from build123d import *

# Parameters (mm, degrees)
SKETCH_2_R          = 8.5
SKETCH_2_R_2        = 8
CUT_EXTRUDE_1_DEPTH = 28
CUT_EXTRUDE_START   = 2
SKETCH_3_R          = 8
SKETCH_3_R_2        = 7
CUT_EXTRUDE_2_DEPTH = 2


with BuildPart() as part:
    # 草图1 → 旋转1 (revolve)
    with BuildSketch(Plane.XY, mode=Mode.PRIVATE) as revolve_1_sk:
        Polygon((0, 0), (0, 13), (3, 13), (3, 8.5), (70, 8.5), (70, 0), align=None)
    revolve(revolve_1_sk.sketch.rotate(Axis((0, 0, 0), (1, 0, 0)), 90), axis=Axis((0, 0, 0), (1, 0, 0)))

    # 草图2 → 切除-拉伸1 (cut)
    with BuildSketch(Plane(origin=(70, 0, 0), x_dir=(0, 0, -1), z_dir=(1, 0, 0))):
        with Locations(Location((0, 0, 0), (0, 0, 180))):
            Circle(SKETCH_2_R)
        Circle(SKETCH_2_R_2, mode=Mode.SUBTRACT)
    extrude(amount=-CUT_EXTRUDE_1_DEPTH, mode=Mode.SUBTRACT)

    # 草图3 → 切除-拉伸2 (cut)
    with BuildSketch(Plane(origin=(42, 0, 0), x_dir=(0, 0, -1), z_dir=(1, 0, 0)).offset(CUT_EXTRUDE_START)):
        Circle(SKETCH_3_R)
        Circle(SKETCH_3_R_2, mode=Mode.SUBTRACT)
    extrude(amount=-CUT_EXTRUDE_2_DEPTH, mode=Mode.SUBTRACT)


solid = part.part
Input: part model. Units: mm. Frame: model coordinates. A direction names the side the tool comes from. Give positions to 0.01 mm unless a question says otherwise; leave off trailing zeros. Loops run counter-clockwise (first coordinate to the right, second up) from the corner with the lowest first, then second, coordinate; pieces in that order, holes last. Notation, with made-up numbers: M 56,-26 L 108,-26 A15 ccw 108,-19 Z; hole C 76,55 d9. An arc over 180 degrees is marked long. Use one line per item in the form item = value.
1. First-contact query: pin 1 (3 mm diameter, centred on x = 26, y = 6, fed in from -Z); pin 2 (10 mm diameter, centred on x = 16, z = 4.5, fed in from -Y); pin 3 (3 mm diameter, centred on x = 56.5, y = 4, fed in from -Z). Flat tips, straight axial feed; report the tip coordinate or a pass-through.
Numbers:
pin_1 = -7.21
pin_2 = -8.5
pin_3 = -7.6
2. Reachability of faces 4 (the face through (3, 8.5, 2.7)), 5 (the face through (1.521, 7.91, -10.316)), 6 (the face through (42, -7, 2)) from +Z, -Z, +X, -X, +Y, -Y: full face, straight path, thin tool, end or side. Return the list, or none.
Numbers:
face_4 = +X
face_5 = +X, -X
face_6 = none
3. Pull-direction query (X, two-part tool) for faces 1 (the face through (70, 0, 0)), 2 (the face through (43.014, -2.681, -6.466)), 3 (the face through (22.773, -8.428, -1.107)); classes: released by +X, released by -X, zero draft, split by the parting line, or undercut.
Numbers:
face_1 = released by +X
face_2 = undercut
face_3 = zero draft
4. Section query D-D, the plane x = 49. Return the cut outline in (y, z).
Numbers:
outline = C 0,0 d16
5. Section query A-A, the plane z = 0. Return the cut outline in (x, y), and give its area (4 significant figures).
Numbers:
outline = M 0,-13 L 3,-13 L 3,-8.5 L 42,-8.5 L 42,-7 L 44,-7 L 44,-8 L 70,-8 L 70,8 L 44,8 L 44,7 L 42,7 L 42,8.5 L 3,8.5 L 3,13 L 0,13 Z
area = 1,185 mm²
6. Line query: L1, parallel to X at y = 3.75, z = 11; L2, parallel to Y at x = 63, z = 0.5; L3, parallel to X at y = 7.25, z = -4. Output: solid intervals per line, ascending.
Numbers:
L1 = 0 to 3
L2 = -7.98 to 7.98
L3 = 0 to 42
7. Section query C-C, the plane x = 30.5. Return the cut outline in (y, z), and give its area (3 significant figures).
Numbers:
outline = C 0,0 d17
area = 227 mm²
